Source: CAD feature listing. Evaluate the final solid. Frame: model axes, mm. Coordinates: 2 decimals unless noted, no trailing zeros. Order: outer loops, then holes, each group sorted by start corner. A loop starts at its lowest first (then second) coordinate and runs counter-clockwise, first axis right, second up. Notation, with made-up numbers: (34.5, -2) -> (64.5, -2) arc R30 ccw to (64.5, 34) -> close; hole circle Ø8 at (-5, 59.25). An arc over 180 degrees is marked (long way). Write each question's results on one line, items separated by ' | '. Start each with the question number.
from build123d import *

# Parameters (mm, degrees)
BOSS_EXTRUDE1_DEPTH = 6
FILLET1_R           = 5


with BuildPart() as part:
    # Sketch1 → Boss-Extrude1 (new, symmetric)
    with BuildSketch(Plane.XY):
        Polygon((-60, 0), (60, 0), (60, 10), (35, 50), (35, 60), (-35, 60), (-35, 50), (-60, 10), align=None)
    extrude(amount=BOSS_EXTRUDE1_DEPTH, both=True)

    # Fillet1
    fillet1_edges = [part.edges().sort_by_distance(p)[0] for p in [
        (-35, 60, 0),
        (35, 60, 0),
    ]]
    fillet(fillet1_edges, radius=FILLET1_R)


solid = part.part
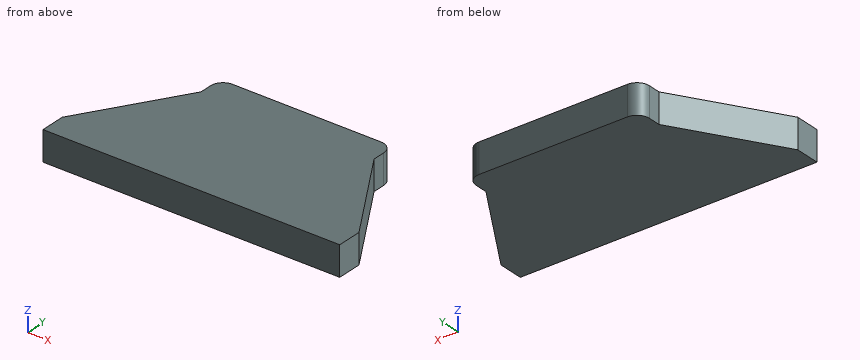
(1) First-contact query: P1, Ø4, axis at y = 53, z = -2, coming from the -X side; P2, Ø4, axis at y = 53.5, z = -1, coming from the +X side; P3, Ø2, axis at y = 25, z = 3.5, coming from the -X side. Flat tips, straight axial feed; report the tip coordinate or a pass-through.
(2) Section C-C on y = 41. Return the cut outline in (x, z) (3 decimals), then the cut area to 3 significant figures.
(3) Section A-A on z = -3.5. Return the cut outline in (x, y), then the cut area to 3 significant figures.
(4) Section B-B on x = -38.5. Return the cut outline in (y, z).
(5) Line query: L1, parallel to X at y = 48, z = 4; L2, parallel to Y at x = 33, z = -3.25; L3, parallel to X at y = 32.5, z = 2. Output: solid intervals per line, ascending.
Results list:
1) P1: stops at x = -35 | P2: stops at x = 35 | P3: stops at x = -51.25
2) outline: (-40.625, -6) -> (40.625, -6) -> (40.625, 6) -> (-40.625, 6) -> close | area: 975 mm²
3) outline: (-60, 0) -> (60, 0) -> (60, 10) -> (35, 50) -> (35, 55) arc R5 ccw to (30, 60) -> (-30, 60) arc R5 ccw to (-35, 55) -> (-35, 50) -> (-60, 10) -> close | area: 5,690 mm²
4) outline: (0, -6) -> (44.4, -6) -> (44.4, 6) -> (0, 6) -> close
5) L1: x = -36.25 to 36.25 | L2: y = 0 to 59 | L3: x = -45.94 to 45.94
